The figure shows three views and two pictorial views of one solid part (mm, origin at its lowest corner). Answer the questions. A direction names the side the tool comes from. Give positions to 0.01 mm unless a question says otherwise; leave off trailing zeros. Loops run counter-clockwise (first coordinate to the right, second up) from the corner with the lowest first, then second, coordinate; pieces in that order, holes last. Notation, with made-up numbers: (-0.5, 30) - (42.5, 30) arc R15 cw to (42.5, 59) - close; hole circle Ø8 at (82, 53.25). An arc over 180 degrees is marked (long way). Write each question's results on one line, items separated by ' | '.
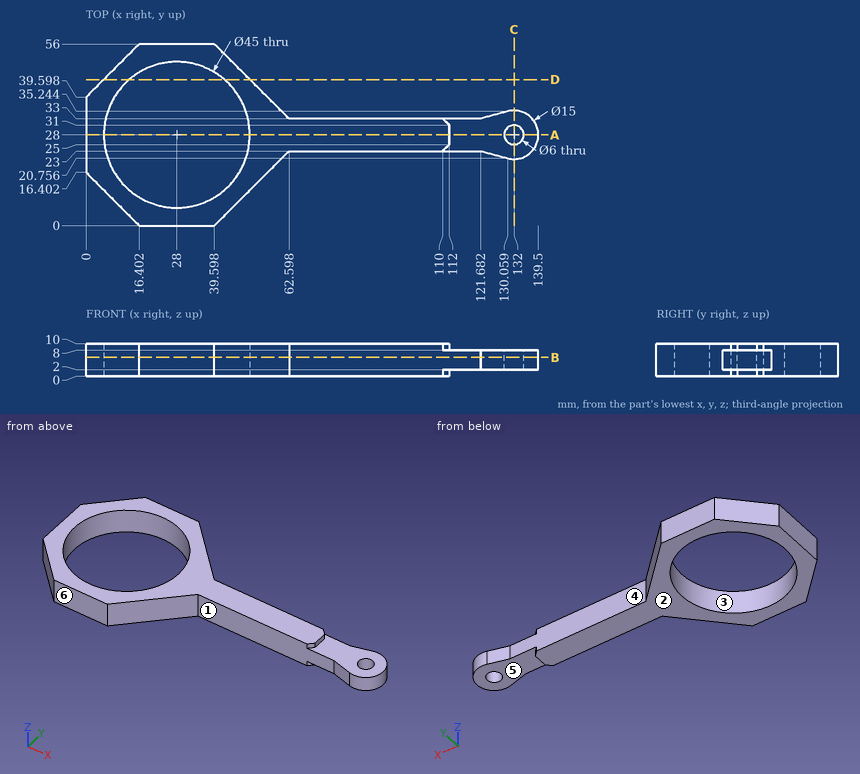
Item 1: A cutting plane is placed at A-A, the plane y = 28. Determine the outline of the cut face in (x, z), plus the area to 3 significant figures.
Values found:
outline: (0, 0) - (5.5, 0) - (5.5, 10) - (0, 10) - close; (50.5, 0) - (112, 0) - (112, 2) - (129, 2) - (129, 8) - (112, 8) - (112, 10) - (50.5, 10) - close; (135, 2) - (139.5, 2) - (139.5, 8) - (135, 8) - close | area: 799 mm²
Item 2: For a pull along Y with two mould halves and no side action, classify the marked faces 3, 4, 5 and 6 as released by +Y, released by -Y, zero draft, split by the parting line, or undercut.
Values found:
face 3: undercut | face 4: released by +Y | face 5: zero draft | face 6: released by -Y
Item 3: A cutting plane is placed at D-D, the plane y = 45. Determine the outline of the cut face in (x, z).
Values found:
outline: (5.4, 0) - (13.26, 0) - (13.26, 10) - (5.4, 10) - close; (42.74, 0) - (50.6, 0) - (50.6, 10) - (42.74, 10) - close
Item 4: Flat-ended cylindrical pins translate along their axes: P1, Ø2, axis at x = 65.5, z = 1.5, coming from the +Y side; P2, Ø5, axis at x = 78.5, z = 5, coming from the -Y side; P3, Ø5.5, axis at x = 132, y = 28, coming from the -Z side; P4, Ø16.5, axis at x = 128, y = 27.5, coming from the -Z side. Find the tip coordinate at first contact, or state that the pin passes through.
Values found:
P1: stops at y = 33 | P2: stops at y = 23 | P3: passes through | P4: stops at z = 2
Item 5: For the marked faces 1 and 2, determine the directions among +Z, -Z, +X, -X, +Y, -Y from which every point of the face is accessible in a straight line to the end or side of a thin tool.
Values found:
face 1: +Z, -Z, -Y | face 2: -Z, +X, -X, +Y, -Y
Item 6: Find the intervals of material crossed by line 1 along Y through (x, z) = (28, 3.75); line 2 along Y through (x, z) = (132, 6.4); line 3 along Y through (x, z) = (110, 2), in increasing order. Write a range as [from, to].
Values found:
line 1: y = [0, 5.5], [50.5, 56] | line 2: y = [20.5, 25], [31, 35.5] | line 3: y = [23, 33]
Item 7: A cutting plane is placed at B-B, the plane z = 5.75. Determine the outline of the cut face in (x, y) (1 decimal).
Values found:
outline: (0, 16.4) - (16.4, 0) - (39.6, 0) - (62.6, 23) - (121.7, 23) - (130.1, 20.8) arc R7.5 ccw (long way) to (130.1, 35.2) - (121.7, 33) - (62.6, 33) - (39.6, 56) - (16.4, 56) - (0, 39.6) - close; hole circle Ø45 at (28, 28); hole circle Ø6 at (132, 28)
Item 8: A cutting plane is placed at C-C, the plane x = 132. Determine the outline of the cut face in (y, z), plus the area to 3 significant figures.
Values found:
outline: (20.5, 2) - (25, 2) - (25, 8) - (20.5, 8) - close; (31, 2) - (35.5, 2) - (35.5, 8) - (31, 8) - close | area: 54.0 mm²
